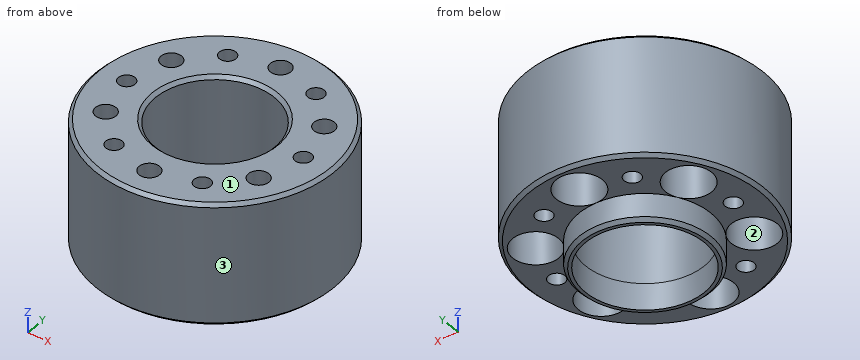
from build123d import *

# Parameters (mm, degrees)
SKETCH_1_R          = 18
SKETCH_1_R_2        = 1.55
SKETCH_1_R_3        = 9
EXTRUDE_1_DEPTH     = 18.4
SKETCH_4_R          = 3.5
CUT_EXTRUDE_1_DEPTH = 7
EXTRUDE_START       = 4
SKETCH_5_R          = 10
SKETCH_5_R_2        = 9
EXTRUDE_2_DEPTH     = 4
HOLE_WIZARD_M3_1_D  = 2.5
CHAMFER_1_SIZE      = 0.5


with BuildPart() as part:
    # 草图1 → 凸台-拉伸1 (new body)
    with BuildSketch(Plane.XY):
        with Locations(Location((0, 0, 0), (0, 0, 180))):
            Circle(SKETCH_1_R)
        with Locations(Location((0, 13.5, 0), (0, 0, 180))):
            Circle(SKETCH_1_R_2, mode=Mode.SUBTRACT)
        with Locations(Location((11.691342951, 6.75, 0), (0, 0, 180))):
            Circle(SKETCH_1_R_2, mode=Mode.SUBTRACT)
        with Locations(Location((11.691342951, -6.75, 0), (0, 0, 180))):
            Circle(SKETCH_1_R_2, mode=Mode.SUBTRACT)
        with Locations(Location((0, -13.5, 0), (0, 0, 180))):
            Circle(SKETCH_1_R_2, mode=Mode.SUBTRACT)
        with Locations(Location((-11.691342951, -6.75, 0), (0, 0, 180))):
            Circle(SKETCH_1_R_2, mode=Mode.SUBTRACT)
        with Locations(Location((-11.691342951, 6.75, 0), (0, 0, 180))):
            Circle(SKETCH_1_R_2, mode=Mode.SUBTRACT)
        with Locations(Location((0, 0, 0), (0, 0, 180))):
            Circle(SKETCH_1_R_3, mode=Mode.SUBTRACT)
    extrude(amount=EXTRUDE_1_DEPTH)

    # 草图4 → 切除-拉伸1 (cut)
    with BuildSketch(Plane.XY):
        with Locations((0, 13.5)):
            Circle(SKETCH_4_R)
        with Locations((11.691342951, 6.75)):
            Circle(SKETCH_4_R)
        with Locations((11.691342951, -6.75)):
            Circle(SKETCH_4_R)
        with Locations((0, -13.5)):
            Circle(SKETCH_4_R)
        with Locations((-11.691342951, -6.75)):
            Circle(SKETCH_4_R)
        with Locations((-11.691342951, 6.75)):
            Circle(SKETCH_4_R)
    extrude(amount=CUT_EXTRUDE_1_DEPTH, mode=Mode.SUBTRACT)

    # 草图5 → 凸台-拉伸2 (add)
    with BuildSketch(Plane(origin=(0, 0, 0), x_dir=(-1, 0, 0), z_dir=(0, 0, -1)).offset(EXTRUDE_START)):
        with Locations(Location((0, 0, 0), (0, 0, 209.999869527))):
            Circle(SKETCH_5_R)
        Circle(SKETCH_5_R_2, mode=Mode.SUBTRACT)
    extrude(amount=-EXTRUDE_2_DEPTH)

    # M3 螺纹孔1 (through all)
    with Locations(Plane.XY.offset(18.4)):
        with Locations((13.5, 0), (6.75, -11.691342951), (-6.75, -11.691342951), (-13.5, 0), (-6.75, 11.691342951), (6.75, 11.691342951)):
            Hole(HOLE_WIZARD_M3_1_D / 2)

    # 倒角1
    chamfer_1_edges = [part.edges().sort_by_distance(p)[0] for p in [
        (18, 0, 0),
        (9, 0, 18.4),
        (18, 0, 18.4),
        (-8.660265424, 4.999980279, -4),
    ]]
    chamfer(chamfer_1_edges, length=CHAMFER_1_SIZE)


solid = part.part
Work out the finished part from the listing and answer in its coordinate system (mm). Face numbers are marked on the shaded views. Give positions to 0.01 mm unless a question says otherwise; leave off trailing zeros. Use a Markdown table: item, result. Add a question column.
1) Each of these flat-tipped pins is pushed along its axis until it touches: P1, Ø1, axis at x = 1.5, y = 11.5, coming from the -Z side; P2, Ø2.5, axis at x = 0, y = 13.5, coming from the +Z side; P3, Ø1, axis at x = -0.5, z = -1, coming from the -Y side; P4, Ø3, axis at x = 6.75, y = -11.69, coming from the -Z side. Where does it stop, or does it pass through?
2) Consider line 1 along Y through (x, z) = (0, 12.75); line 2 along Y through (x, z) = (0, -1.2); line 3 along Y through (x, z) = (11, 7.5). Determine where each line is inside the solid, lowest interval first.
3) For a pull along X with two mould halves and no side action, classify the marked faces 1, 2 and 3 as +X half, -X half, draft (parallel to the pull), parting line (faces both ways), or undercut.
4) The part is cut by section A-A, the plane z = 4. Count the separate pieces of the cut face and the enclosed holes in it, plus the area to 3 significant figures.
Reported:
| question | item | result |
|---|---|---|
| 1 | P1 | stops at z = 7 |
| 1 | P2 | passes through |
| 1 | P3 | stops at y = -10 |
| 1 | P4 | stops at z = 0 |
| 2 | line 1 | y = -18 to -15.05, -11.95 to -9, 9 to 11.95, 15.05 to 18 |
| 2 | line 2 | y = -10 to -9, 9 to 10 |
| 2 | line 3 | y = -14.25 to -8.14, -5.36 to 5.36, 8.14 to 14.25 |
| 3 | face 1 | draft |
| 3 | face 2 | undercut |
| 3 | face 3 | parting line |
| 4 | separate pieces | 1 |
| 4 | enclosed holes | 13 |
| 4 | area | 503 mm^2 |
